Part model, mm, in its own coordinate system. A direction names the side the tool comes from. Give positions to 0.01 mm unless a question says otherwise; leave off trailing zeros. Order: outer loops, then holes, each group sorted by start corner. A loop starts at its lowest first (then second) coordinate and runs counter-clockwise, first axis right, second up. Notation, with made-up numbers: (-4, 61) - (49, 61) arc R32 ccw to (49, 93) - close; hole circle Ø10 at (3.5, -10.5). An arc over 180 degrees is marked (long way). One line per item, written item: value.
```python
from build123d import *

# Parameters (mm, degrees)
BOSS_EXTRUDE1_DEPTH      = 9.525
BOSS_EXTRUDE1_DEPTH_BACK = 9.525
SKETCH1_R                = 9.525
BOSS_EXTRUDE2_DEPTH      = 12.7
BOSS_EXTRUDE2_DEPTH_BACK = 12.7
BOSS_EXTRUDE2_START      = -9.525
SKETCH2_R                = 3.175
CUT_EXTRUDE1_DEPTH       = 19.513272266
CUT_EXTRUDE1_DEPTH_BACK  = 19.513272266
SKETCH3_R                = 4.7625


with BuildPart() as part:
    # Sketch1 → Boss-Extrude1 (new, two sides: drawn at the far end of the back side and taken through both)
    with BuildSketch(Plane.XY.offset(-BOSS_EXTRUDE1_DEPTH_BACK)):
        Circle(SKETCH1_R)
    extrude(amount=BOSS_EXTRUDE1_DEPTH + BOSS_EXTRUDE1_DEPTH_BACK)

    # Sketch2 → Boss-Extrude2 (add, two sides: drawn at the far end of the back side and taken through both)
    with BuildSketch(Plane.XY.offset(9.525).offset(BOSS_EXTRUDE2_START - BOSS_EXTRUDE2_DEPTH_BACK)):
        Circle(SKETCH2_R)
    extrude(amount=BOSS_EXTRUDE2_DEPTH + BOSS_EXTRUDE2_DEPTH_BACK)

    # Sketch3 → Cut-Extrude1 (cut, two sides: drawn at the far end of the back side and taken through both)
    with BuildSketch(Plane(origin=(0, 0, 0), x_dir=(0, 0, -1), z_dir=(1, 0, 0)).offset(-CUT_EXTRUDE1_DEPTH_BACK)):
        Circle(SKETCH3_R)
    extrude(amount=CUT_EXTRUDE1_DEPTH + CUT_EXTRUDE1_DEPTH_BACK, mode=Mode.SUBTRACT)


solid = part.part
```
1) Mould opens along Y. For faces 1 (the cylindrical face through (-0.133, 4.016, -2.56)), 2 (the cylindrical face through (-0.69, -3.1, 11.09)), 3 (the flat face through (4, 0, 9.525)) say: released by +Y, released by -Y, zero draft, split by the parting line, or undercut.
Outcome:
face 1: undercut
face 2: split by the parting line
face 3: zero draft
2) Cut at B-B, the plane x = 0. Give the cut face in (y, z) (1 decimal), then the cut area to 3 significant figures.
Outcome:
outline: (-9.5, -9.5) - (-3.2, -9.5) - (-3.2, -12.7) - (3.2, -12.7) - (3.2, -9.5) - (9.5, -9.5) - (9.5, 9.5) - (3.2, 9.5) - (3.2, 12.7) - (-3.2, 12.7) - (-3.2, 9.5) - (-9.5, 9.5) - close; hole circle Ø9.5 at (0, 0)
area: 332 mm^2
3) Pin check, flat tips, straight feed: pin 1 (2 mm diameter, centred on y = 7.5, z = 8, fed in from -X); pin 2 (1.5 mm diameter, centred on x = 1.5, y = 4, fed in from +Z) (3 decimals); pin 3 (8.5 mm diameter, centred on y = 0, z = 0, fed in from -X); pin 4 (1.5 mm diameter, centred on x = -6, z = 1, fed in from +Y). Stop position of each tip, or through.
Outcome:
pin 1: stops at x = -6.96
pin 2: stops at z = 9.525
pin 3: passes through
pin 4: stops at y = 7.95
4) Which spindle directions (+Z, -Z, +X, -X, +Y, -Y) get a long thin tool onto all of the face, cutting with end or side? Do faces 4 (the flat face through (4, 0, -9.525)), 5 (the flat face through (0, 0, -12.7)). Say none if no direction does.
Outcome:
face 4: -Z
face 5: -Z, +X, -X, +Y, -Y
5) Cut at C-C, the plane y = -3.75. Give the cut face in (x, z) (3 decimals).
Outcome:
outline: (-8.756, -9.525) - (8.756, -9.525) - (8.756, -2.936) - (-8.756, -2.936) - close; (-8.756, 2.936) - (8.756, 2.936) - (8.756, 9.525) - (-8.756, 9.525) - close
6) Cut at A-A, the plane y = 0. Give the cut face in (x, z) (1 decimal), then the cut area to 3 significant figures.
Outcome:
outline: (-9.5, -9.5) - (-3.2, -9.5) - (-3.2, -12.7) - (3.2, -12.7) - (3.2, -9.5) - (9.5, -9.5) - (9.5, -4.8) - (-9.5, -4.8) - close; (-9.5, 4.8) - (9.5, 4.8) - (9.5, 9.5) - (3.2, 9.5) - (3.2, 12.7) - (-3.2, 12.7) - (-3.2, 9.5) - (-9.5, 9.5) - close
area: 222 mm^2
7) Cut at D-D, the plane z = 8.5. Give the cut face in (x, y) (3 decimals).
Outcome:
outline: circle Ø19.05 at (0, 0)
8) Drill centre lines: line 1 along Z through (x, y) = (-0.5, 0); line 2 along Z through (x, y) = (-4.5, 0) (1 decimal); line 3 along Z through (x, y) = (8, 5) (3 decimals). Where is each one in solid material? Low to high. Write a range as from..to.
Outcome:
line 1: z = -12.7..-4.76, 4.76..12.7
line 2: z = -9.5..-4.8, 4.8..9.5
line 3: z = -9.525..9.525
